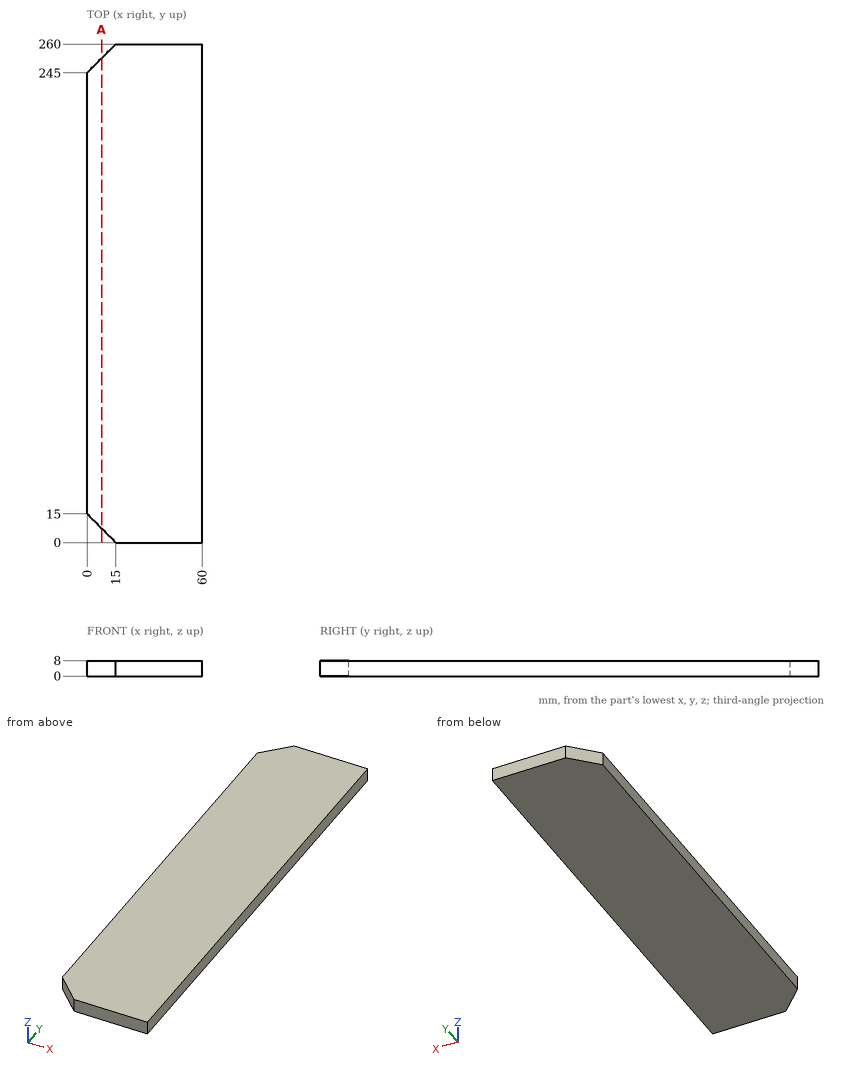
Here's the drawing with two shaded views (mm, measured from the low corner). I have some questions. Coordinates: 2 decimals unless noted, no trailing zeros. Loops run counter-clockwise (first coordinate to the right, second up) from the corner with the lowest first, then second, coordinate; pieces in that order, holes last. Notation, with made-up numbers: (85, 86.25) -> (97, 86.25) arc R22 ccw to (97, 121.25) -> close; hole circle Ø5 at (8, -5.75). An arc over 180 degrees is marked (long way). Put each result on its own line as item: value. Start each with the question number.
Q1. I want a section at A-A (x = 7.5). Write out the boundary of the cut face in (y, z).
Q2. If I drill on line 1 (Y direction, x = 6, z = 3.25); line 2 (Y direction, x = 12, z = 5.5); line 3 (X direction, y = 247, z = 0.5), over which ranges is the centre line in solid material (lowest first)? Write a range as [from, to].
Q3. I'm going to push a flat-ended pin straight in: P1, Ø1, axis at x = 12, z = 4.5, coming from the +Y side. Where does the tip first touch, or does it pass through?
Taken from the geometry:
1. outline: (7.5, 0) -> (252.5, 0) -> (252.5, 8) -> (7.5, 8) -> close
2. line 1: y = [9, 251]
2. line 2: y = [3, 257]
2. line 3: x = [2, 60]
3. P1: stops at y = 257.5
